from build123d import *

# Parameters (mm, degrees)
SKETCH_1_R             = 7.5
EXTRUDE_1_DEPTH        = 12
SKETCH_2_R             = 8
EXTRUDE_2_DEPTH        = 60
SKETCH_3_R             = 10.5
EXTRUDE_3_DEPTH        = 315
EXTRUDE_START          = 12
SKETCH_4_R             = 7.5
EXTRUDE_4_DEPTH        = 12
SKETCH_5_R             = 7
EXTRUDE_5_DEPTH        = 32
SKETCH_6_W             = 4.707373346
SKETCH_6_H             = 4.483082856
CUT_EXTRUDE_1_DEPTH    = 30
HOLE_WIZARD_M8_1_D     = 6.8
HOLE_WIZARD_M8_1_DEPTH = 19.75
HOLE_WIZARD_M8_1_TIP   = 2.042926105
HOLE_WIZARD_M4_1_D     = 3.3


with BuildPart() as part:
    # 草图1 → 凸台-拉伸1 (new body)
    with BuildSketch(Plane.XY):
        Circle(SKETCH_1_R)
    extrude(amount=EXTRUDE_1_DEPTH)

    # 草图2 → 凸台-拉伸2 (add)
    with BuildSketch(Plane(origin=(0, 0, 0), x_dir=(-1, 0, 0), z_dir=(0, 0, -1))):
        Circle(SKETCH_2_R)
    extrude(amount=EXTRUDE_2_DEPTH)

    # 草图3 → 凸台-拉伸3 (add)
    with BuildSketch(Plane(origin=(0, 0, -60), x_dir=(-1, 0, 0), z_dir=(0, 0, -1))):
        Circle(SKETCH_3_R)
    extrude(amount=EXTRUDE_3_DEPTH)

    # 草图4 → 凸台-拉伸4 (add)
    with BuildSketch(Plane(origin=(0, 0, -375), x_dir=(-1, 0, 0), z_dir=(0, 0, -1)).offset(EXTRUDE_START)):
        Circle(SKETCH_4_R)
    extrude(amount=-EXTRUDE_4_DEPTH)

    # 草图5 → 凸台-拉伸5 (add)
    with BuildSketch(Plane(origin=(0, 0, -387), x_dir=(-1, 0, 0), z_dir=(0, 0, -1))):
        Circle(SKETCH_5_R)
    extrude(amount=EXTRUDE_5_DEPTH)

    # 草图6 → 切除-拉伸1 (cut)
    with BuildSketch(Plane(origin=(0, 0, -419), x_dir=(-1, 0, 0), z_dir=(0, 0, -1))):
        with Locations((0, 7)):
            Rectangle(SKETCH_6_W, SKETCH_6_H)
    extrude(amount=-CUT_EXTRUDE_1_DEPTH, mode=Mode.SUBTRACT)

    # M8 螺纹孔1
    with Locations(Plane.XY.offset(12)):
        with Locations((0, 0)):
            Hole(HOLE_WIZARD_M8_1_D / 2, depth=HOLE_WIZARD_M8_1_DEPTH)
            with Locations((0, 0, -(HOLE_WIZARD_M8_1_DEPTH + HOLE_WIZARD_M8_1_TIP / 2))):  # 118° drill point
                Cone(0, HOLE_WIZARD_M8_1_D / 2, HOLE_WIZARD_M8_1_TIP, mode=Mode.SUBTRACT)

    # M4 螺纹孔1 (through all)
    with Locations(Plane(origin=(-0.010980736, 7.499991962, 6.6634249), x_dir=(0.999998928208, 0.001464098146, 0), z_dir=(-0.001464098146, 0.999998928208, 0))):
        with Locations((0, 0)):
            Hole(HOLE_WIZARD_M4_1_D / 2)


solid = part.part
Work out the finished part from the listing and answer in its coordinate system (mm). A direction names the side the tool comes from. Give positions to 0.01 mm unless a question says otherwise; leave off trailing zeros. Order: outer loops, then holes, each group sorted by start corner. A loop starts at its lowest first (then second) coordinate and runs counter-clockwise, first axis right, second up. Notation, with made-up numbers: (21, -31.75) -> (43, -31.75) arc R16 cw to (43, -16.75) -> close; hole circle Ø3 at (17.25, -6). An arc over 180 degrees is marked (long way). One line per item, written item: value.
Item 1: Straight lines are drawn through the part: probe 1 along Y at (x, z) = (0, 3); probe 2 along Y at (x, z) = (0, -2.25); probe 3 along X at (y, z) = (-6.75, -109.5). For each, find the intervals that lie inside material, in ascending order.
Answer sheet:
probe 1: -7.5 to -3.4, 3.4 to 7.5
probe 2: -8 to -3.4, 3.4 to 8
probe 3: -8.04 to 8.04
Item 2: Find section A-A, the plane z = -88. Give the vertices of the cut face in (x, y), plus the area to 3 significant figures.
Answer sheet:
outline: circle Ø21 at (0, 0)
area: 346 mm²
Item 3: A tool of negligible diameter and unlimited length cuts with its end or side. For faces 1 (the cylindrical face through (7.493, 0.33, -381.084)), 2 (the flat face through (2, -3, 12)), 3 (the flat face through (-5, -6, 0)), from which of +Z, -Z, +X, -X, +Y, -Y can it reach the whole face along a straight path? Write none if from no direction.
Answer sheet:
face 1: -Z
face 2: +Z, +X, -X, +Y, -Y
face 3: +Z
Item 4: Find section B-B, the plane z = -22.5. Give the vertices of the cut face in (x, y).
Answer sheet:
outline: circle Ø16 at (0, 0)
Item 5: Flat-ended cylindrical pins translate along their axes: P1, Ø2, axis at x = 7, z = -370, coming from the -Y side; P2, Ø2.5, axis at x = 0.5, z = -397, coming from the +Y side; P3, Ø2, axis at y = 2, z = -67, coming from the +X side. Find the tip coordinate at first contact, or state that the pin passes through.
Answer sheet:
P1: y = -8.62
P2: y = 4.76
P3: x = 10.45
